Check sheet for the drawn part. Datum: minimum x, y, z corner. Units: mm. Coordinates: 2 decimals unless noted, no trailing zeros. Write each loop counter-clockwise with the first axis right and the second up, starting at its lowest first coordinate (ties: lowest second). Pieces come first, ordered by that corner, then holes. Notation, with made-up numbers: M 33.25,-29.5 L 79.25,-29.5 A17 ccw 79.25,1.5 Z; hole C -6,23 d1. An arc over 180 degrees is marked long. Answer as a JSON object with one key per item and string values. Group by question number.
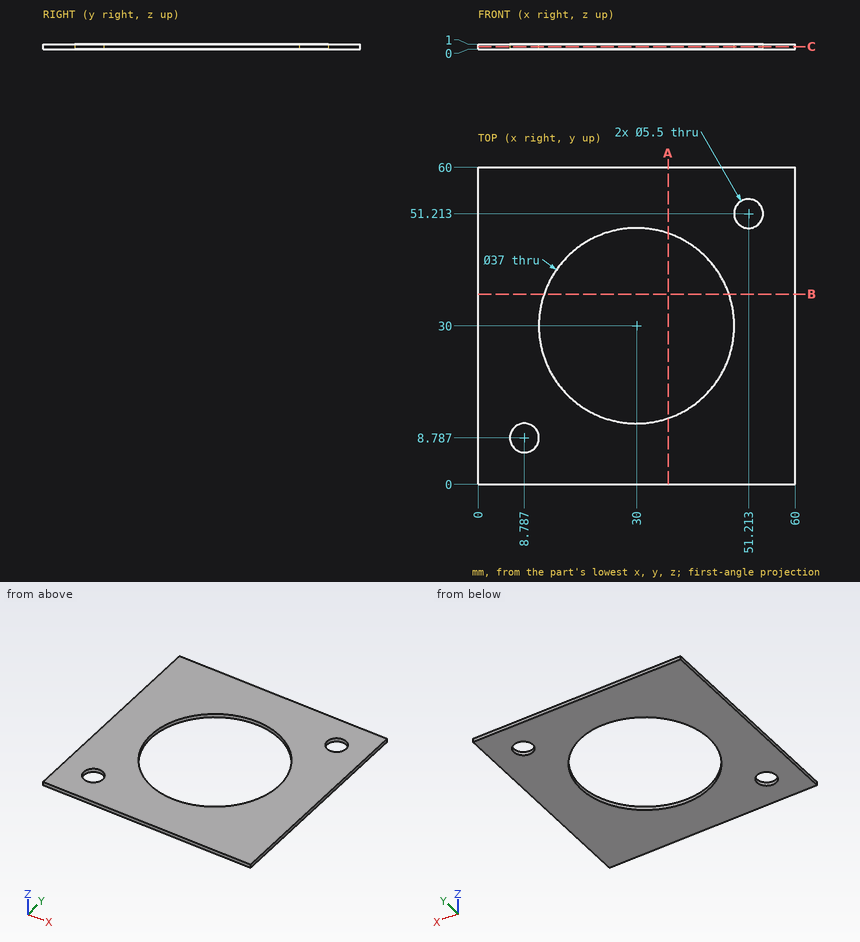
1) Material ranges on probe 1 along Y at (x, z) = (29, 0.6); probe 2 along X at (y, z) = (46, 0.9); probe 3 along X at (y, z) = (19, 0.6) (1 decimal), recorded low to high. Write a range as [from, to].
2) Section check C-C (z = 0.5). Record the cut outline in (x, y).
3) Go/stop test with a flat-tipped pin: pin 1 Ø4 at (x, y) = (36.5, 44) entering from -Z. Record where the tip stops, or that it passes through.
4) Section check A-A (x = 36). Record the cut outline in (y, z), then the cut area to 3 significant figures.
Entries:
{
 "1": {"probe 1": "[0, 11.53], [48.47, 60]", "probe 2": "[0, 20.71], [39.29, 60]", "probe 3": "[0, 15.1], [44.9, 60]"},
 "2": {"outline": "M 0,0 L 60,0 L 60,60 L 0,60 Z; hole C 8.79,8.79 d5.5; hole C 30,30 d37; hole C 51.21,51.21 d5.5"},
 "3": {"pin 1": "through"},
 "4": {"outline": "M 0,0 L 12.5,0 L 12.5,1 L 0,1 Z; M 47.5,0 L 60,0 L 60,1 L 47.5,1 Z", "area": "25.0 mm^2"}
}
